Geometry: final body of the model. Coordinates: model frame, mm. Face numbers are marked on the shaded views. Give positions to 0.01 mm unless a question says otherwise; leave off trailing zeros. Order: outer loops, then holes, each group sorted by start corner. A loop starts at its lowest first (then second) coordinate and runs counter-clockwise, first axis right, second up. Notation, with made-up numbers: (53, 12.5) - (73, 12.5) arc R15 cw to (73, 36.5) - close; hole circle Ø2 at (0, -11.75). An arc over 180 degrees is marked (long way). One line per item, written item: value.
```python
from build123d import *

# Parameters (mm, degrees)
SKETCH_1_W         = 23
SKETCH_1_H         = 30
EXTRUDE_1_DEPTH    = 10
CHAMFER_1_SIZE     = 5
HOLE_WIZARD_M8_1_D = 6.8


with BuildPart() as part:
    # 草图1 → 凸台-拉伸1 (new body)
    with BuildSketch(Plane.XY):
        Rectangle(SKETCH_1_W, SKETCH_1_H)
    extrude(amount=EXTRUDE_1_DEPTH)

    # 倒角1
    chamfer_1_edges = [part.edges().sort_by_distance(p)[0] for p in [
        (11.5, 15, 5),
        (11.5, -15, 5),
    ]]
    chamfer(chamfer_1_edges, length=CHAMFER_1_SIZE)

    # M8 螺纹孔1 (through all)
    with Locations(Plane(origin=(0, 0, 0), x_dir=(-1, 0, 0), z_dir=(0, 0, -1))):
        with Locations((-1.5, 0)):
            Hole(HOLE_WIZARD_M8_1_D / 2)


solid = part.part
```
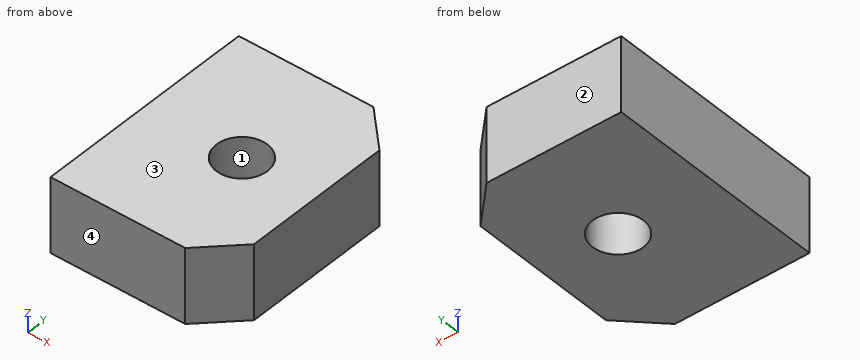
1) Section B-B, the plane y = 0. Return loops of the section in (x, z).
Answers below:
outline: (-11.5, 0) - (-1.9, 0) - (-1.9, 10) - (-11.5, 10) - close; (4.9, 0) - (11.5, 0) - (11.5, 10) - (4.9, 10) - close
2) Section A-A, the plane z = 3. Return loops of the section in (x, y), then the cut area to 3 significant figures.
Answers below:
outline: (-11.5, -15) - (6.5, -15) - (11.5, -10) - (11.5, 10) - (6.5, 15) - (-11.5, 15) - close; hole circle Ø6.8 at (1.5, 0)
area: 629 mm^2
3) Section C-C, the plane x = 1.5. Return loops of the section in (y, z).
Answers below:
outline: (-15, 0) - (-3.4, 0) - (-3.4, 10) - (-15, 10) - close; (3.4, 0) - (15, 0) - (15, 10) - (3.4, 10) - close
4) Section D-D, the plane y = -10.5. Return loops of the section in (x, z).
Answers below:
outline: (-11.5, 0) - (11, 0) - (11, 10) - (-11.5, 10) - close
5) Material intervals for line 1 along Y through (x, z) = (1.5, 5.5); line 2 along Y through (x, z) = (3, 5.5); line 3 along X through (y, z) = (2, 6), sorted ascending.
Answers below:
line 1: -15 to -3.4, 3.4 to 15
line 2: -15 to -3.05, 3.05 to 15
line 3: -11.5 to -1.25, 4.25 to 11.5
6) Mould query, pull axis Y, two halves, no side actions, for the marked faces 1, 2, 3 and 4. Classes: released by +Y, released by -Y, zero draft, split by the parting line, or undercut.
Answers below:
face 1: undercut
face 2: released by +Y
face 3: zero draft
face 4: released by -Y
